Part model, mm, in its own coordinate system. Coordinates: 2 decimals unless noted, no trailing zeros. Order: outer loops, then holes, each group sorted by start corner. A loop starts at its lowest first (then second) coordinate and runs counter-clockwise, first axis right, second up.
1) Cut at A-A (x = 4.5). List the corners of the cut face in (y, z).
2) Pin check, flat tip, straight feed: pin 1 Ø2 at (x, y) = (38.25, 16.5) entering from +Z. Stop position of the tip, or through.
3) Wall check: L1, parallel to Y at x = 38.25, z = 0.25; L2, parallel to Y at x = 34.5, z = 0.9; L3, parallel to X at y = 7, z = 0.6. Give the ranges that are in metal, low to high.
4) Cut at D-D (x = 38.25). List the corners of the cut face in (y, z), and give its area (3 significant figures).
5) Cut at B-B (z = 0.55). List the corners of the cut face in (x, y), and give its area (3 significant figures).
6) Cut at C-C (y = -13). List the corners of the cut face in (x, z).
7) Mould opens along X. For faces 1 (the cylindrical face through (-37.309, -15.024, 0.493)), 2 (the flat face through (-10, -18, 1)) say: +X half, -X half, draft (parallel to the pull), parting line (faces both ways), or undercut.
```python
from build123d import *

# Parameters (mm, degrees)
SKETCH1_W           = 83.5
SKETCH1_H           = 42
SKETCH1_R           = 1.75
SKETCH1_W_2         = 72.5
SKETCH1_H_2         = 31
BOSS_EXTRUDE1_DEPTH = 1
FILLET1_R           = 1


with BuildPart() as part:
    # Sketch1 → Boss-Extrude1 (new body)
    with BuildSketch(Plane.XY):
        Rectangle(SKETCH1_W, SKETCH1_H)
        with Locations((-38.25, 16.5)):
            Circle(SKETCH1_R, mode=Mode.SUBTRACT)
        with Locations((38.25, 16.5)):
            Circle(SKETCH1_R, mode=Mode.SUBTRACT)
        with Locations((38.25, -16.5)):
            Circle(SKETCH1_R, mode=Mode.SUBTRACT)
        with Locations((-38.25, -16.5)):
            Circle(SKETCH1_R, mode=Mode.SUBTRACT)
        with Locations((0, 18)):
            Circle(SKETCH1_R, mode=Mode.SUBTRACT)
        with Locations((0, -18)):
            Circle(SKETCH1_R, mode=Mode.SUBTRACT)
        Rectangle(SKETCH1_W_2, SKETCH1_H_2, mode=Mode.SUBTRACT)
    extrude(amount=BOSS_EXTRUDE1_DEPTH)

    # Fillet1
    fillet1_edges = [part.edges().sort_by_distance(p)[0] for p in [
        (-36.25, 15.5, 0.5),
        (-36.25, -15.5, 0.5),
        (36.25, -15.5, 0.5),
        (36.25, 15.5, 0.5),
    ]]
    fillet(fillet1_edges, radius=FILLET1_R)


solid = part.part
```
Geometry check:
1. outline: (-21, 0) - (-15.5, 0) - (-15.5, 1) - (-21, 1) - close; (15.5, 0) - (21, 0) - (21, 1) - (15.5, 1) - close
2. pin 1: passes through
3. L1: y = -21 to -18.25, -14.75 to 14.75, 18.25 to 21
3. L2: y = -21 to -15.5, 15.5 to 21
3. L3: x = -41.75 to -36.25, 36.25 to 41.75
4. outline: (-21, 0) - (-18.25, 0) - (-18.25, 1) - (-21, 1) - close; (-14.75, 0) - (14.75, 0) - (14.75, 1) - (-14.75, 1) - close; (18.25, 0) - (21, 0) - (21, 1) - (18.25, 1) - close
4. area: 35.0 mm2
5. outline: (-41.75, -21) - (41.75, -21) - (41.75, 21) - (-41.75, 21) - close; hole circle Ø3.5 at (-38.25, -16.5); hole circle Ø3.5 at (-38.25, 16.5); hole (-36.25, -14.5) arc R1 ccw to (-35.25, -15.5) - (35.25, -15.5) arc R1 ccw to (36.25, -14.5) - (36.25, 14.5) arc R1 ccw to (35.25, 15.5) - (-35.25, 15.5) arc R1 ccw to (-36.25, 14.5) - close; hole circle Ø3.5 at (0, -18); hole circle Ø3.5 at (0, 18); hole circle Ø3.5 at (38.25, -16.5); hole circle Ø3.5 at (38.25, 16.5)
5. area: 1,200 mm2
6. outline: (-41.75, 0) - (-36.25, 0) - (-36.25, 1) - (-41.75, 1) - close; (36.25, 0) - (41.75, 0) - (41.75, 1) - (36.25, 1) - close
7. face 1: undercut
7. face 2: draft
